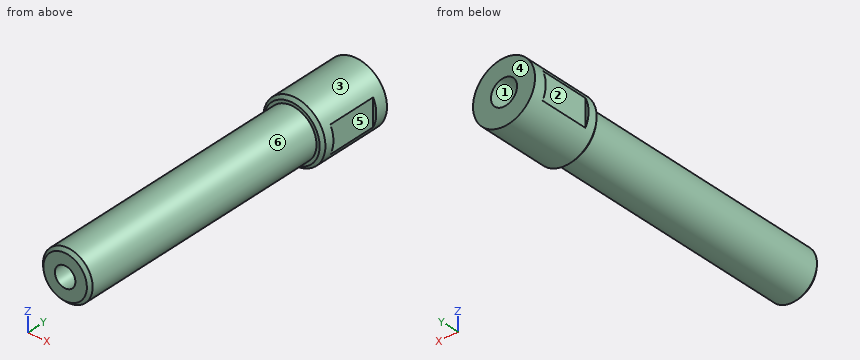
```python
from build123d import *

# Parameters (mm, degrees)
SKETCH1_R             = 4
BOSS_EXTRUDE1_DEPTH   = 42.3
SKETCH2_R             = 5
BOSS_EXTRUDE2_DEPTH   = 12
M5_TAPPED_HOLE1_D     = 4.2
M5_TAPPED_HOLE1_DEPTH = 12.4
M5_TAPPED_HOLE1_TIP   = 1.2618073
M4_TAPPED_HOLE1_D     = 3.3
M4_TAPPED_HOLE1_DEPTH = 10.1
M4_TAPPED_HOLE1_TIP   = 0.991420021
SKETCH5_W             = 1
SKETCH5_H             = 8
CUT_EXTRUDE1_DEPTH    = 5
CHAMFER1_SIZE         = 0.5


with BuildPart() as part:
    # Sketch1 → Boss-Extrude1 (new body)
    with BuildSketch(Plane(origin=(0, 0, 0), x_dir=(1, 0, 0), z_dir=(0, 1, 0))):
        with Locations(Location((0, 0, 0), (0, 0, 270))):
            Circle(SKETCH1_R)
    extrude(amount=BOSS_EXTRUDE1_DEPTH)

    # Sketch2 → Boss-Extrude2 (add)
    with BuildSketch(Plane(origin=(0, 42.3, 0), x_dir=(1, 0, 0), z_dir=(0, 1, 0))):
        with Locations(Location((0, 0, 0), (0, 0, 270))):
            Circle(SKETCH2_R)
    extrude(amount=BOSS_EXTRUDE2_DEPTH)

    # M5 Tapped Hole1
    with Locations(Plane.ZX.offset(54.3)):
        with Locations((0, 0)):
            Hole(M5_TAPPED_HOLE1_D / 2, depth=M5_TAPPED_HOLE1_DEPTH)
            with Locations((0, 0, -(M5_TAPPED_HOLE1_DEPTH + M5_TAPPED_HOLE1_TIP / 2))):  # 118° drill point
                Cone(0, M5_TAPPED_HOLE1_D / 2, M5_TAPPED_HOLE1_TIP, mode=Mode.SUBTRACT)

    # M4 Tapped Hole1
    with Locations(Plane(origin=(0, 0, 0), x_dir=(0, 0, -1), z_dir=(0, -1, 0))):
        with Locations((0, 0)):
            Hole(M4_TAPPED_HOLE1_D / 2, depth=M4_TAPPED_HOLE1_DEPTH)
            with Locations((0, 0, -(M4_TAPPED_HOLE1_DEPTH + M4_TAPPED_HOLE1_TIP / 2))):  # 118° drill point
                Cone(0, M4_TAPPED_HOLE1_D / 2, M4_TAPPED_HOLE1_TIP, mode=Mode.SUBTRACT)

    # Sketch5 → Cut-Extrude1 (cut, symmetric)
    with BuildSketch(Plane.XY):
        with Locations((-5, 48.3)):
            Rectangle(SKETCH5_W, SKETCH5_H)
        with Locations((5, 48.3)):
            Rectangle(SKETCH5_W, SKETCH5_H)
    extrude(amount=CUT_EXTRUDE1_DEPTH, both=True, mode=Mode.SUBTRACT)

    # Chamfer1
    chamfer1_edges = [part.edges().sort_by_distance(p)[0] for p in [
        (0, 0, -4),
        (0, 42.3, -5),
    ]]
    chamfer(chamfer1_edges, length=CHAMFER1_SIZE)


solid = part.part
```
For this review, take the finished solid that the model builds, in its own axes (mm). Face numbers are marked on the shaded views. A direction names the side the tool comes from. Coordinates: 2 decimals unless noted, no trailing zeros. Write each loop counter-clockwise with the first axis right and the second up, starting at its lowest first coordinate (ties: lowest second). Pieces come first, ordered by that corner, then holes.
(1) Wall thickness on probe 1 along X at (y, z) = (49.25, 0); probe 2 along X at (y, z) = (3.75, 0); probe 3 along Y at (x, z) = (-2.5, -3.75): over which ranges is each line inside the solid? List them lowest first.
(2) Add section B-B on y = 38.5. Give the boundary of the cut face in (x, z), then the cut area to 3 significant figures.
(3) Tool access review of the marked faces 4, 5 and 6: name each direction out of +Z, -Z, +X, -X, +Y, -Y from which nothing blocks a thin tool from reaching the whole face with its end or side.
(4) For pin 1 Ø1.3 at (y, z) = (46.5, -1) entering from -X; pin 2 Ø0.6 at (x, z) = (-5, 0.5) entering from -Y; pin 3 Ø4 at (y, z) = (25, -2) entering from +X, all flat-tipped, find the tip position at first contact; note any pin that passes through.
(5) The part is to be moulded in two halves that separate along Z. For the marked faces 1, 2 and 3, say which applies: +Z half, -Z half, draft (parallel to the pull), parting line (faces both ways), or undercut.
(6) Add section A-A on y = 47.5. Give the boundary of the cut face in (x, z), then the cut area to 3 significant figures.
Answer sheet:
1. probe 1: x = -4.5 to -2.1, 2.1 to 4.5
1. probe 2: x = -4 to -1.65, 1.65 to 4
1. probe 3: y = 42.31 to 54.3
2. outline: circle Ø8 at (0, 0)
2. area: 50.3 mm2
3. face 4: +Z, -Z, +X, -X, +Y
3. face 5: +Z, -Z, +X
3. face 6: -Y
4. pin 1: stops at x = -4.5
4. pin 2: stops at y = 42.52
4. pin 3: stops at x = 4
5. face 1: undercut
5. face 2: draft
5. face 3: parting line
6. outline: (-4.5, -2.18) arc R5 ccw to (4.5, -2.18) - (4.5, 2.18) arc R5 ccw to (-4.5, 2.18) - close; hole circle Ø4.2 at (0, 0)
6. area: 61.7 mm2
